The listing builds one solid part. Answer for the finished solid, in the listing's coordinates (mm). Give positions to 0.01 mm unless a question says otherwise; leave off trailing zeros. Order: outer loops, then holes, each group sorted by start corner. A loop starts at its lowest first (then second) coordinate and runs counter-clockwise, first axis right, second up. Notation, with made-up numbers: (-18, 79.5) -> (35, 79.5) arc R23 cw to (35, 110.5) -> close; hole circle Ø4 at (22.25, 16.5). An arc over 180 degrees is marked (long way). One line per question, with ' | ' between items. Start each with the question number.
```python
from build123d import *

# Parameters (mm, degrees)
SKETCH_1_W      = 60
SKETCH_1_H      = 60
SKETCH_1_R      = 18.5
SKETCH_1_R_2    = 2.75
EXTRUDE_1_DEPTH = 1


with BuildPart() as part:
    # 草图1 → 凸台-拉伸1 (new body)
    with BuildSketch(Plane.XY):
        with Locations((30, 30)):
            Rectangle(SKETCH_1_W, SKETCH_1_H)
        with Locations((30, 30)):
            Circle(SKETCH_1_R, mode=Mode.SUBTRACT)
        with Locations((8.786796564, 8.786796564)):
            Circle(SKETCH_1_R_2, mode=Mode.SUBTRACT)
        with Locations((51.213203436, 51.213203436)):
            Circle(SKETCH_1_R_2, mode=Mode.SUBTRACT)
    extrude(amount=EXTRUDE_1_DEPTH)


solid = part.part
```
(1) Given P1, Ø12, axis at x = 36.5, y = 14, coming from the -Z side, flat-ended and moving along its own axis, determine where the tip first touches the part or whether it passes through.
(2) The part is cut by section C-C on z = 0.55. Determine the outline of the cut face in (x, y), plus the area to 3 significant figures.
(3) The part is cut by section A-A on x = 30. Determine the outline of the cut face in (y, z), plus the area to 3 significant figures.
(4) Determine the mould class of faces 1 (the face through (6.76, 10.645, 0.493)), 2 (the face through (15.32, 18.74, 0.49)), 3 (the face through (16, 44, 1)) for opening direction X: pulls with the +X half, pulls with the -X half, needs draft (parallel to the pull), parting line crosses it, or undercut.
(5) Consider line 1 (Y direction, x = 30, z = 0.6); line 2 (X direction, y = 7.5, z = 0.25); line 3 (X direction, y = 13, z = 0.8). Determine where each line is inside the solid, lowest interval first.
Result sheet:
1) P1: stops at z = 0
2) outline: (0, 0) -> (60, 0) -> (60, 60) -> (0, 60) -> close; hole circle Ø5.5 at (8.79, 8.79); hole circle Ø37 at (30, 30); hole circle Ø5.5 at (51.21, 51.21) | area: 2,480 mm^2
3) outline: (0, 0) -> (11.5, 0) -> (11.5, 1) -> (0, 1) -> close; (48.5, 0) -> (60, 0) -> (60, 1) -> (48.5, 1) -> close | area: 23.0 mm^2
4) face 1: undercut | face 2: undercut | face 3: needs draft
5) line 1: y = 0 to 11.5, 48.5 to 60 | line 2: x = 0 to 6.36, 11.22 to 60 | line 3: x = 0 to 22.7, 37.3 to 60
